CAD build for the part. Positions are in the model's coordinates, mm. A direction names the side the tool comes from. Coordinates: 2 decimals unless noted, no trailing zeros. Loops run counter-clockwise (first coordinate to the right, second up) from the corner with the lowest first, then second, coordinate; pieces in that order, holes last.
1) Saw through at C-C, the plane z = -11.5. Write the cut outline in (x, y).
2) Wall check: line 1 along X through (y, z) = (-25, -27); line 2 along Z through (x, y) = (57.5, -10); line 3 along Z through (x, y) = (41, -9.5). Give the ranges that are in metal, low to high.
3) Pin check, flat tips, straight feed: pin 1 Ø2 at (x, z) = (42, 9.5) entering from -Y; pin 2 Ø3 at (x, y) = (29, -10) entering from -Z; pin 3 Ø1.5 at (x, y) = (29, -23) entering from +Z. Stop position of each tip, or through.
4) Saw through at B-B, the plane x = 36. Write the cut outline in (y, z).
5) Which spindle directions (+Z, -Z, +X, -X, +Y, -Y) get a long thin tool onto all of the face, cutting with end or side? Do faces 1 (the flat face through (34, -35, 15)), 2 (the flat face through (30, -13, 0)), 3 (the flat face through (46, -30, -15)), 4 (the flat face through (8, -25, -85)). Say none if no direction does.
6) Saw through at D-D, the plane z = -27. Write the cut outline in (x, y).
7) Two-plate mould, pull along Y, no slides. Class faces 5 (the cylindrical face through (8, -30, -65)), 6 (the flat face through (34, -25, 15)), 7 (the cylindrical face through (63, -30, 10)), 8 (the flat face through (62.8, -29.6, 35)): +Y half, -Y half, draft (parallel to the pull), parting line (faces both ways), or undercut.
8) Saw through at A-A, the plane y = -48. Write the cut outline in (x, z), and give its area (4 significant figures).
```python
from build123d import *

# Parameters (mm, degrees)
BASE_BLOCK_SKETCH_W       = 70
BASE_BLOCK_SKETCH_H       = 60
BASE_BLOCK_60X70X15_DEPTH = 15
UPPER_ROUND_LUG_DEPTH     = 15
UPPER_SLOT_10MM_DEPTH     = 15
TOP_PLATE_SKETCH_W        = 78
TOP_PLATE_SKETCH_H        = 60
TOP_PLATE_78MM_DEPTH      = 15
RADIUS_CUT_SKETCH_R       = 30
RADIUS_CUT_DEPTH          = 15
LOWER_START               = -50
LOWER_LUG_50MM_DEPTH      = 50
SUPPORT_RIB_10MM_REACH    = 132.001
RIB_SKETCH_WALL_W         = 322.001968056
RIB_SKETCH_WALL_H         = 10


with BuildPart() as part:
    # Base Block Sketch → Base Block 60x70x15 (new body)
    with BuildSketch(Plane(origin=(0, 0, 0), x_dir=(0, 0, -1), z_dir=(1, 0, 0))):
        with Locations((35, -30)):
            Rectangle(BASE_BLOCK_SKETCH_W, BASE_BLOCK_SKETCH_H)
    extrude(amount=BASE_BLOCK_60X70X15_DEPTH)

    # Upper Lug Sketch → Upper Round Lug (add)
    with BuildSketch(Plane.ZY):
        with BuildLine():
            Line((-70, 0), (-70, -60))
            ThreePointArc((-70, -60), (-100, -30), (-70, 0))
        make_face()
    extrude(amount=-UPPER_ROUND_LUG_DEPTH)

    # Upper Slot Sketch → Upper Slot 10mm (cut)
    with BuildSketch(Plane(origin=(15, 0, 0), x_dir=(0, 0, -1), z_dir=(1, 0, 0))):
        with BuildLine():
            Line((70, -25), (99.580398915, -25))
            ThreePointArc((99.580398915, -25), (104.580398915, -30), (99.580398915, -35))
            Line((99.580398915, -35), (70, -35))
            ThreePointArc((70, -35), (65, -30), (70, -25))
        make_face()
    extrude(amount=-UPPER_SLOT_10MM_DEPTH, mode=Mode.SUBTRACT)

    # Top Plate Sketch → Top Plate 78mm (add)
    with BuildSketch(Plane.XY):
        with Locations((39, -30)):
            Rectangle(TOP_PLATE_SKETCH_W, TOP_PLATE_SKETCH_H)
    extrude(amount=-TOP_PLATE_78MM_DEPTH)

    # Radius Cut Sketch → Radius Cut (cut)
    with BuildSketch(Plane.XY):
        with Locations((78, -30)):
            Circle(RADIUS_CUT_SKETCH_R)
    extrude(amount=-RADIUS_CUT_DEPTH, mode=Mode.SUBTRACT)

    # Lower Lug Sketch → Lower Lug 50mm (add)
    with BuildSketch(Plane(origin=(0, 0, -15), x_dir=(-1, 0, 0), z_dir=(0, 0, -1)).offset(LOWER_START)):
        with BuildLine():
            Line((-78, -60), (-78, -45))
            ThreePointArc((-78, -45), (-63, -30), (-78, -15))
            Line((-78, -15), (-78, 0))
            ThreePointArc((-78, 0), (-48, -30), (-78, -60))
        make_face()
    extrude(amount=LOWER_LUG_50MM_DEPTH)

    # Rib Sketch wall → Support Rib 10mm (add, up to next)
    with BuildSketch(Plane(origin=(24.366985862, -30, 17.5), x_dir=(0.812232862067, 0, 0.583333333334), z_dir=(-0.583333333334, 0, 0.812232862067)), mode=Mode.PRIVATE) as support_rib_10mm_sk1:
        Rectangle(RIB_SKETCH_WALL_W, RIB_SKETCH_WALL_H)
    support_rib_10mm_tool1 = extrude(support_rib_10mm_sk1.sketch, amount=-SUPPORT_RIB_10MM_REACH, mode=Mode.PRIVATE) - part.part
    add(support_rib_10mm_tool1.solids().sort_by_distance((24.366985862, -30, 17.5))[0])


solid = part.part
```
Data:
1. outline: (0, -60) - (78, -60) - (78, -45) arc R15 cw to (78, -15) - (78, 0) - (0, 0) - close
2. line 1: x = 0 to 15
2. line 2: z = -15 to 35
2. line 3: z = -15 to 0
3. pin 1: stops at y = -35
3. pin 2: stops at z = -15
3. pin 3: stops at z = 0
4. outline: (-60, -15) - (0, -15) - (0, 0) - (-25, 0) - (-25, 25.85) - (-35, 25.85) - (-35, 0) - (-60, 0) - close
5. face 1: +Z, -X, -Y
5. face 2: +Z, -X, +Y
5. face 3: -Z, +X, +Y, -Y
5. face 4: -Z, +X, -X
6. outline: (0, -60) - (15, -60) - (15, 0) - (0, 0) - close
7. face 5: undercut
7. face 6: +Y half
7. face 7: undercut
7. face 8: draft
8. outline: (0, -94) - (15, -94) - (15, -15) - (78, -15) - (78, 35) - (54, 35) - (54, 0) - (0, 0) - close
8. area: 3,195 mm2
